Can you work these out from the model? Positions are in its coordinate system, mm. Coordinates: 2 decimals unless noted, no trailing zeros. Write each loop counter-clockwise with the first axis right and the second up, starting at its lowest first coordinate (ties: lowest second). Pieces come first, ordered by that corner, then holes. Notation, with made-up numbers: M 89,28 L 101,28 A20 ccw 101,44 Z; hole C -33,70.25 d6. An arc over 180 degrees is marked long. Use one line per item in the form item = value. Start each with the question number.
```python
from build123d import *

# Parameters (mm, degrees)
SKETCH1_R           = 9
SKETCH1_R_2         = 3.25
BOSS_EXTRUDE1_DEPTH = 3
CHAMFER1_SIZE       = 0.5


with BuildPart() as part:
    # Sketch1 → Boss-Extrude1 (new body)
    with BuildSketch(Plane.XY):
        Circle(SKETCH1_R)
        Circle(SKETCH1_R_2, mode=Mode.SUBTRACT)
    extrude(amount=BOSS_EXTRUDE1_DEPTH)

    # Chamfer1
    chamfer1_edges = [part.edges().sort_by_distance(p)[0] for p in [
        (-9, 0, 0),
        (-9, 0, 3),
        (-3.25, 0, 0),
        (-3.25, 0, 3),
    ]]
    chamfer(chamfer1_edges, length=CHAMFER1_SIZE)


solid = part.part
```
1) Suppose I cut it at C-C on z = 1.7. Please give me the cut outline in (x, y).
2) If we mould it in two halves opening along Y, with no side actions, what happens to faces 1 (the face through (-2.579, -1.978, 1.486)), 2 (the face through (-1.172, 8.923, 1.486)), 3 (the face through (4, -2, 3))? For each: +Y half, -Y half, draft (parallel to the pull), parting line (faces both ways), or undercut.
3) Will these pins go through, and if not, where does the flat tip stop? pin 1 Ø1.5 at (y, z) = (4, 0.5) entering from +X; pin 2 Ø1.5 at (x, z) = (5, 1) entering from +Y; pin 3 Ø1.5 at (y, z) = (-2, 2) entering from -X.
4) Suppose I cut it at A-A on x = 0. Please give me the cut outline in (y, z).
5) Please list where these lines run through material, in increasing order: line 1 (Y direction, x = 0, z = 1.75); line 2 (X direction, y = 2.5, z = 0.4); line 3 (X direction, y = 1.5, z = 1.5).
Computed values:
q1.outline = C 0,0 d18; hole C 0,0 d6.5
q2.face_1 = undercut
q2.face_2 = parting line
q2.face_3 = draft
q3.pin_1 = 8.39
q3.pin_2 = 7.93
q3.pin_3 = -8.91
q4.outline = M -9,0.5 L -8.5,0 L -3.75,0 L -3.25,0.5 L -3.25,2.5 L -3.75,3 L -8.5,3 L -9,2.5 Z; M 3.25,0.5 L 3.75,0 L 8.5,0 L 9,0.5 L 9,2.5 L 8.5,3 L 3.75,3 L 3.25,2.5 Z
q5.line_1 = -9 to -3.25, 3.25 to 9
q5.line_2 = -8.54 to -2.23, 2.23 to 8.54
q5.line_3 = -8.87 to -2.88, 2.88 to 8.87
